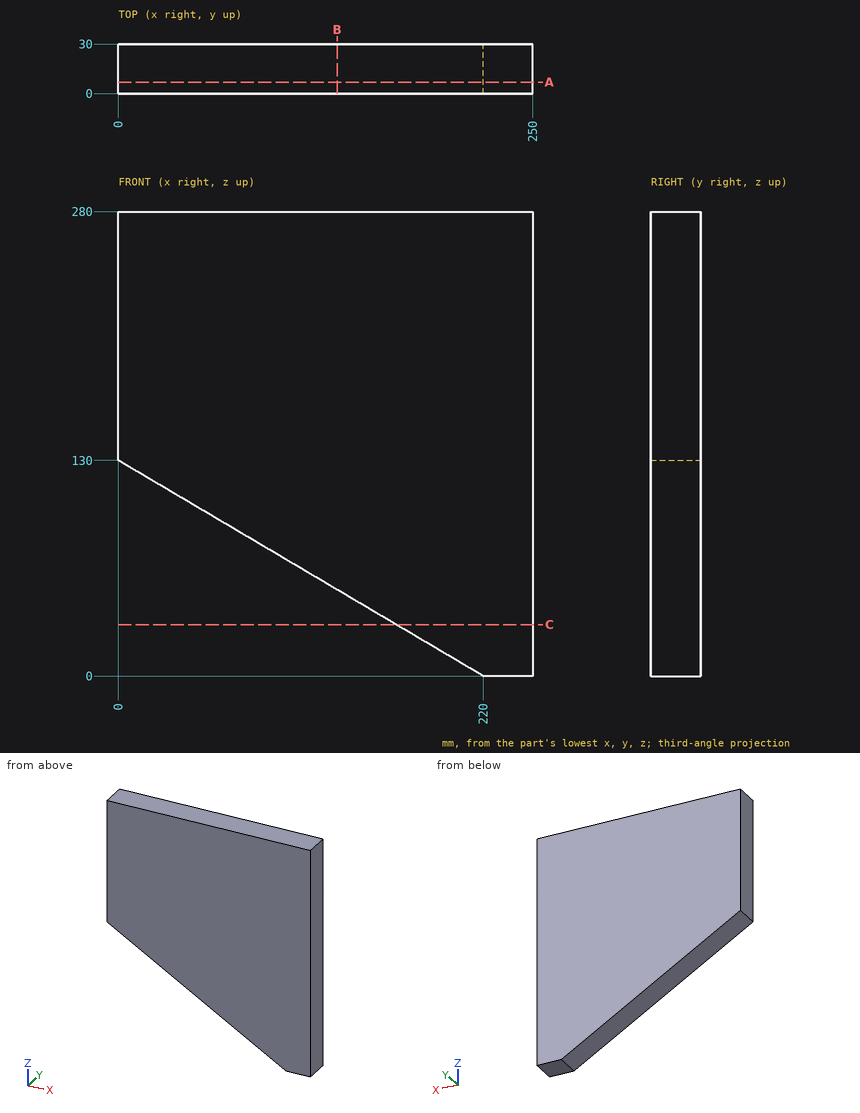
Design review of the part shown in the three views and the two pictorial views. Dimensions are in mm from the part's minimum x, y and z. Give positions to 0.01 mm unless a question says otherwise; leave off trailing zeros. Loops run counter-clockwise (first coordinate to the right, second up) from the corner with the lowest first, then second, coordinate; pieces in that order, holes last. Notation, with made-up numbers: (-22, 88.25) - (9, 88.25) arc R10 cw to (9, 98.25) - close; hole circle Ø1 at (83.25, 65.25). An arc over 180 degrees is marked (long way). Use CSV: the item, a comma, the result in double quotes. Start each with the question number.
1. Add section A-A (y = 7). State the section outline as (x, z) points.
2. Add section B-B (x = 132). State the section outline as (y, z) points.
3. Add section C-C (z = 31). State the section outline as (x, y) points, plus the area to 3 significant figures.
4. Insertion check: P1, Ø3, axis at x = 105, y = 19, coming from the -Z side. The pin has a flat end and moves straight along its axis. Give the tip position at first contact, or say it passes through.
5. Wall thickness on L1, parallel to Z at x = 139.5, y = 19.5; L2, parallel to X at y = 26.5, z = 59; L3, parallel to Z at x = 134.5, y = 7: over which ranges is each line inside the solid? List them lowest first.
Results found:
1,outline,"(0, 130) - (220, 0) - (250, 0) - (250, 280) - (0, 280) - close"
2,outline,"(0, 52) - (30, 52) - (30, 280) - (0, 280) - close"
3,outline,"(167.54, 0) - (250, 0) - (250, 30) - (167.54, 30) - close"
3,area,"2,470 mm²"
4,P1,"stops at z = 67.07"
5,L1,"z = 47.57 to 280"
5,L2,"x = 120.15 to 250"
5,L3,"z = 50.52 to 280"
